from build123d import *

# Parameters (mm, degrees)
FLANGE_PLATE_SKETCH_R       = 11.665
FLANGE_PLATE_SKETCH_R_2     = 52.5
FLANGE_PLATE_SKETCH_R_3     = 40.5
FLANGE_PLATE_DEPTH          = 12
HOUSING_BOSS_SKETCH_R       = 52.5
HOUSING_BOSS_SKETCH_R_2     = 40.5
BEARING_HOUSING_BOSS_DEPTH  = 38
BOLT_BOSS_SKETCH_R          = 23.665
BOLT_BOSS_SKETCH_R_2        = 11.665
BOLT_BOSSES_2X_DEPTH        = 13
FLANGE_RELIEF_POCKETS_DEPTH = 3


with BuildPart() as part:
    # Flange Plate Sketch → Flange Plate (new body)
    # profile 1 of 3: a face of its own
    with BuildSketch(Plane(origin=(0, 0, 0), x_dir=(1, 0, 0), z_dir=(0, 1, 0))):
        with BuildLine():
            ThreePointArc((-17.301, -49.56738241), (-52.5, 0), (-17.301, 49.56738241))
            Line((-17.301, 49.56738241), (-95.298631714, 22.343087709))
            ThreePointArc((-95.298631714, 22.343087709), (-111.165, 0), (-95.298631714, -22.343087709))
            Line((-95.298631714, -22.343087709), (-17.301, -49.56738241))
        make_face()
        with Locations(Location((-87.5, 0, 0), (0, 0, 270))):
            Circle(FLANGE_PLATE_SKETCH_R, mode=Mode.SUBTRACT)
    # profile 2 of 3: a face of its own
    with BuildSketch(Plane(origin=(0, 0, 0), x_dir=(1, 0, 0), z_dir=(0, 1, 0))):
        with BuildLine():
            Line((95.298631714, 22.343087709), (17.301, 49.56738241))
            ThreePointArc((17.301, 49.56738241), (42.805096075, 30.396936523), (52.5, 0))
            ThreePointArc((52.5, 0), (42.805096075, -30.396936523), (17.301, -49.56738241))
            Line((17.301, -49.56738241), (95.298631714, -22.343087709))
            ThreePointArc((95.298631714, -22.343087709), (111.165, 0), (95.298631714, 22.343087709))
        make_face()
        with Locations(Location((87.5, 0, 0), (0, 0, 270))):
            Circle(FLANGE_PLATE_SKETCH_R, mode=Mode.SUBTRACT)
    # profile 3 of 3: a face of its own
    with BuildSketch(Plane(origin=(0, 0, 0), x_dir=(1, 0, 0), z_dir=(0, 1, 0))):
        Circle(FLANGE_PLATE_SKETCH_R_2)
        with Locations(Location((0, 0, 0), (0, 0, 270))):
            Circle(FLANGE_PLATE_SKETCH_R_3, mode=Mode.SUBTRACT)
    extrude(amount=FLANGE_PLATE_DEPTH)

    # Housing Boss Sketch → Bearing Housing Boss (add)
    with BuildSketch(Plane(origin=(0, 12, 0), x_dir=(1, 0, 0), z_dir=(0, 1, 0))):
        with Locations(Location((0, 0, 0), (0, 0, 109.241031138))):
            Circle(HOUSING_BOSS_SKETCH_R)
        with Locations(Location((0, 0, 0), (0, 0, 270))):
            Circle(HOUSING_BOSS_SKETCH_R_2, mode=Mode.SUBTRACT)
    extrude(amount=BEARING_HOUSING_BOSS_DEPTH)

    # Bolt Boss Sketch → Bolt Bosses 2x (add)
    # profile 1 of 2: a face of its own
    with BuildSketch(Plane(origin=(0, 12, 0), x_dir=(1, 0, 0), z_dir=(0, 1, 0))):
        with Locations(Location((87.5, 0, 0), (0, 0, 70.758968862))):
            Circle(BOLT_BOSS_SKETCH_R)
        with Locations(Location((87.5, 0, 0), (0, 0, 270))):
            Circle(BOLT_BOSS_SKETCH_R_2, mode=Mode.SUBTRACT)
    # profile 2 of 2: a face of its own
    with BuildSketch(Plane(origin=(0, 12, 0), x_dir=(1, 0, 0), z_dir=(0, 1, 0))):
        with Locations(Location((-87.5, 0, 0), (0, 0, 109.241031138))):
            Circle(BOLT_BOSS_SKETCH_R)
        with Locations(Location((-87.5, 0, 0), (0, 0, 270))):
            Circle(BOLT_BOSS_SKETCH_R_2, mode=Mode.SUBTRACT)
    extrude(amount=BOLT_BOSSES_2X_DEPTH)

    # Relief Pocket Sketch → Flange Relief Pockets (cut)
    with BuildSketch(Plane(origin=(0, 12, 0), x_dir=(1, 0, 0), z_dir=(0, 1, 0))):
        with BuildLine():
            Line((71.809327621, 27.364302024), (49.82603874, 35.037349549))
            ThreePointArc((49.82603874, 35.037349549), (46.470783868, 34.048587089), (46.332927596, 30.553392944))
            ThreePointArc((46.332927596, 30.553392944), (55.5, 0), (46.332927596, -30.553392944))
            ThreePointArc((46.332927596, -30.553392944), (46.470783868, -34.048587089), (49.82603874, -35.037349549))
            Line((49.82603874, -35.037349549), (71.809327621, -27.364302024))
            ThreePointArc((71.809327621, -27.364302024), (73.795133067, -24.922702734), (72.507464694, -22.050988869))
            ThreePointArc((72.507464694, -22.050988869), (60.835, 0), (72.507464694, 22.050988869))
            ThreePointArc((72.507464694, 22.050988869), (73.795133067, 24.922702734), (71.809327621, 27.364302024))
        make_face()
        with BuildLine():
            Line((-71.809327621, -27.364302024), (-49.82603874, -35.037349549))
            ThreePointArc((-49.82603874, -35.037349549), (-46.470783868, -34.048587089), (-46.332927596, -30.553392944))
            ThreePointArc((-46.332927596, -30.553392944), (-55.5, 0), (-46.332927596, 30.553392944))
            ThreePointArc((-46.332927596, 30.553392944), (-46.470783868, 34.048587089), (-49.82603874, 35.037349549))
            Line((-49.82603874, 35.037349549), (-71.809327621, 27.364302024))
            ThreePointArc((-71.809327621, 27.364302024), (-73.795133067, 24.922702734), (-72.507464694, 22.050988869))
            ThreePointArc((-72.507464694, 22.050988869), (-60.835, 0), (-72.507464694, -22.050988869))
            ThreePointArc((-72.507464694, -22.050988869), (-73.795133067, -24.922702734), (-71.809327621, -27.364302024))
        make_face()
    extrude(amount=-FLANGE_RELIEF_POCKETS_DEPTH, mode=Mode.SUBTRACT)


solid = part.part
Verification items for the finished model (mm, model axes). A direction names the side the tool comes from. Give positions to 0.01 mm unless a question says otherwise; leave off trailing zeros. Loops run counter-clockwise (first coordinate to the right, second up) from the corner with the lowest first, then second, coordinate; pieces in that order, holes last. Notation, with made-up numbers: (4.5, 23.5) - (37.5, 23.5) arc R12 cw to (37.5, 33.5) - close; hole circle Ø8 at (18.5, 2). An arc over 180 degrees is marked (long way). Write item = value, one per line. Start each with the question number.
Q1. Cross-section at B-B, the plane z = 0. State how many separate pieces and enclosed holes the cut face has, and give its area (3 significant figures).
Q2. Cross-section at D-D, the plane x = -22. Enter the section's corners in (y, z), and give its area (3 significant figures).
Q3. Cross-section at C-C, the plane y = 5. Enter the section's corners in (x, z) (3 decimals).
Q4. Mould release check, pull along X, two halves, no side actions. Record for faces 4 (the face through (-56.846, 5.916, 35.765)), 5 (the face through (-26, 0, 34)), 6 (the face through (60.837, 10.521, 0.363)): released by +X, released by -X, zero draft, split by the parting line, or undercut.
Q5. Cross-section at A-A, the plane y = 20. Enter the section's corners in (x, z) (3 decimals).
Q6. Depth check by flat-ended pin: P1, Ø6, axis at y = 7, z = 8, coming from the +X side; P2, Ø6, axis at y = 25.5, z = -3.5, coming from the +X side; P3, Ø3, axis at y = 18, z = 21, coming from the +X side; P4, Ø18.5, axis at x = -87.5, z = 0, coming from the +Y side. Enter the tip coordinate at first touch or a pass-through.
Q7. Tool access check on faces 1 (the face through (55.754, 5.916, 36.146)), 2 (the face through (89, 25, 12)), 3 (the face through (53, 12, 0)). Record the directions out of +Z, -Z, +X, -X, +Y, -Y that give a thin tool (end or side, any length) a straight path to the whole face; none if there is none.
Q8. Thickness scan on line 1 (X direction, y = 18, z = 0) (3 decimals); line 2 (X direction, y = 5, z = 0) (3 decimals); line 3 (X direction, y = 24.5, z = -4.5). Record the ranges inside material, lowest first.
Answer key:
q1.separate_pieces = 4
q1.enclosed_holes = 0
q1.area = 2,640 mm^2
q2.outline = (0, -47.93) - (12, -47.93) - (12, -47.67) - (50, -47.67) - (50, -34) - (0, -34) - close; (0, 34) - (50, 34) - (50, 47.67) - (12, 47.67) - (12, 47.93) - (0, 47.93) - close
q2.area = 1,370 mm^2
q3.outline = (-95.299, -22.343) - (-17.301, -49.567) arc R52.5 ccw to (17.301, -49.567) - (95.299, -22.343) arc R23.665 ccw to (95.299, 22.343) - (17.301, 49.567) arc R52.5 ccw to (-17.301, 49.567) - (-95.299, 22.343) arc R23.665 ccw to start; hole circle Ø23.33 at (-87.5, 0); hole circle Ø81 at (0, 0); hole circle Ø23.33 at (87.5, 0)
q4.face_4 = released by -X
q4.face_5 = zero draft
q4.face_6 = undercut
q5.outline = circle Ø47.33 at (-87.5, 0); circle Ø105 at (0, 0); circle Ø47.33 at (87.5, 0); hole circle Ø23.33 at (-87.5, 0); hole circle Ø81 at (0, 0); hole circle Ø23.33 at (87.5, 0)
q6.P1 = 110.63
q6.P2 = 111.16
q6.P3 = 100.91
q6.P4 = through
q7.face_1 = +Z, +X, +Y, -Y
q7.face_2 = +Z, -Z, +X, +Y
q7.face_3 = +Y
q8.line_1 = -111.165 to -99.165, -75.835 to -63.835, -52.5 to -40.5, 40.5 to 52.5, 63.835 to 75.835, 99.165 to 111.165
q8.line_2 = -111.165 to -99.165, -75.835 to -40.5, 40.5 to 75.835, 99.165 to 111.165
q8.line_3 = -110.73 to -98.26, -76.74 to -64.27, -52.31 to -40.25, 40.25 to 52.31, 64.27 to 76.74, 98.26 to 110.73
